Build history of the part. All positions in model axes, mm. A direction names the side the tool comes from. Give positions to 0.01 mm unless a question says otherwise; leave off trailing zeros. Order: outer loops, then holes, each group sorted by start corner. A loop starts at its lowest first (then second) coordinate and runs counter-clockwise, first axis right, second up. Notation, with made-up numbers: M 81.5,-7 L 111.5,-7 A15 cw 111.5,-3 Z; hole C -3,31.5 d6. An arc over 180 degrees is marked long. Answer as CSV lines item,"result".
from build123d import *

# Parameters (mm, degrees)
SKETCH1_W                                           = 37
SKETCH1_H                                           = 27
BOSS_EXTRUDE1_DEPTH                                 = 10
CBORE_FOR_M5_HEX_SOCKET_HEAD_CAP_SCREW1_D           = 5.5
CBORE_FOR_M5_HEX_SOCKET_HEAD_CAP_SCREW1_CBORE_D     = 10
CBORE_FOR_M5_HEX_SOCKET_HEAD_CAP_SCREW1_CBORE_DEPTH = 5.4
M5_TAPPED_HOLE1_D                                   = 4.2
M5_TAPPED_HOLE1_DEPTH                               = 12.4
M5_TAPPED_HOLE1_TIP                                 = 1.2618073
CHAMFER1_SIZE                                       = 2


with BuildPart() as part:
    # Sketch1 → Boss-Extrude1 (new body)
    with BuildSketch(Plane.XY):
        Rectangle(SKETCH1_W, SKETCH1_H)
    extrude(amount=BOSS_EXTRUDE1_DEPTH)

    # CBORE for M5 Hex Socket Head Cap Screw1 (through all)
    with Locations(Plane.XY.offset(10)):
        with Locations((-13, 7.5), (13, 7.5)):
            CounterBoreHole(CBORE_FOR_M5_HEX_SOCKET_HEAD_CAP_SCREW1_D / 2, CBORE_FOR_M5_HEX_SOCKET_HEAD_CAP_SCREW1_CBORE_D / 2, CBORE_FOR_M5_HEX_SOCKET_HEAD_CAP_SCREW1_CBORE_DEPTH)

    # M5 Tapped Hole1
    with Locations(Plane.XY.offset(10)):
        with Locations((0, -2.5)):
            Hole(M5_TAPPED_HOLE1_D / 2, depth=M5_TAPPED_HOLE1_DEPTH)
            with Locations((0, 0, -(M5_TAPPED_HOLE1_DEPTH + M5_TAPPED_HOLE1_TIP / 2))):  # 118° drill point
                Cone(0, M5_TAPPED_HOLE1_D / 2, M5_TAPPED_HOLE1_TIP, mode=Mode.SUBTRACT)

    # Chamfer1
    chamfer1_edges = [part.edges().sort_by_distance(p)[0] for p in [
        (18.5, -13.5, 5),
        (-18.5, -13.5, 5),
        (-18.5, 13.5, 5),
        (18.5, 13.5, 5),
    ]]
    chamfer(chamfer1_edges, length=CHAMFER1_SIZE)


solid = part.part
Item 1: Drop a flat-ended pin along its axis: pin 1 (5 mm diameter, centred on x = 11, y = 7, fed in from +Z). Give the stop position or say it passes through.
Geometry says:
pin 1,"stops at z = 4.6"
Item 2: Band-saw the part on D-D (y = 7.5). Give the cut face in (x, z), and give its area (3 significant figures).
Geometry says:
outline,"M -18.5,0 L -15.75,0 L -15.75,4.6 L -18,4.6 L -18,10 L -18.5,10 Z; M -10.25,0 L 10.25,0 L 10.25,4.6 L 8,4.6 L 8,10 L -8,10 L -8,4.6 L -10.25,4.6 Z; M 15.75,0 L 18.5,0 L 18.5,10 L 18,10 L 18,4.6 L 15.75,4.6 Z"
area,"211 mm2"
Item 3: Band-saw the part on B-B (z = 8.5). Give the cut face in (x, y).
Geometry says:
outline,"M -18.5,-11.5 L -16.5,-13.5 L 16.5,-13.5 L 18.5,-11.5 L 18.5,11.5 L 16.5,13.5 L -16.5,13.5 L -18.5,11.5 Z; hole C -13,7.5 d10; hole C 0,-2.5 d4.2; hole C 13,7.5 d10"
Item 4: 3-axis set-ups, long thin cutter, end or side, ignore diameter. For faces 5 (the flat face through (18, -12, 5)), 6 (the cylindrical face through (-8.23, 9, 7.34)): which of +Z, -Z, +X, -X, +Y, -Y reach the whole face in a straight line?
Geometry says:
face 5,"+Z, -Z, +X, -Y"
face 6,"+Z"
Item 5: Pull direction Y, two halves, no side cores. Call faces 1 (the cylindrical face through (-12.404, 4.815, 2.268)), 2 (the flat face through (-17, -13, 5)), 3 (the flat face through (18.5, 0, 5)), 4 (the cylindrical face through (17.77, 9, 7.34)): released by +Y, released by -Y, zero draft, split by the parting line, or undercut.
Geometry says:
face 1,"undercut"
face 2,"released by -Y"
face 3,"zero draft"
face 4,"undercut"
Item 6: Probe line 1 along X through (y, z) = (9, 5.25); line 2 along X through (y, z) = (8, 5); line 3 along Y through (x, z) = (-13, 5.5). List the from-to ranges inside material, lowest first. Write a range as from..to.
Geometry says:
line 1,"x = -18.5..-17.77, -8.23..8.23, 17.77..18.5"
line 2,"x = -18.5..-17.97, -8.03..8.03, 17.97..18.5"
line 3,"y = -13.5..2.5, 12.5..13.5"
Item 7: Band-saw the part on A-A (y = -2.5). Give the cut face in (x, z), and give its area (3 significant figures).
Geometry says:
outline,"M -18.5,0 L -2.1,0 L -2.1,10 L -18.5,10 Z; M 2.1,0 L 18.5,0 L 18.5,10 L 2.1,10 Z"
area,"328 mm2"
Item 8: Band-saw the part on C-C (x = 0). Give the cut face in (y, z).
Geometry says:
outline,"M -13.5,0 L -4.6,0 L -4.6,10 L -13.5,10 Z; M -0.4,0 L 13.5,0 L 13.5,10 L -0.4,10 Z"
